from build123d import *

# Parameters (mm, degrees)
EXTRUDE_THIN1_DEPTH = 20
CHAMFER1_SIZE       = 0.3
CUT_EXTRUDE1_REACH  = 53.386
CUT_EXTRUDE2_REACH  = 55.39
SKETCH3_R           = 1.75


with BuildPart() as part:
    # Sketch1 → Extrude-Thin1 (new body)
    with BuildSketch(Plane.XY):
        Polygon((0, 45.5), (0, 0), (24.5, 0), (24.5, 5), (5, 5), (5, 45.5), align=None)
    extrude(amount=EXTRUDE_THIN1_DEPTH)

    # Chamfer1
    chamfer1_edges = [part.edges().sort_by_distance(p)[0] for p in [
        (14.75, 5, 20),
        (5, 25.25, 20),
        (2.5, 45.5, 20),
        (0, 22.75, 20),
        (0, 22.75, 0),
        (2.5, 45.5, 0),
        (5, 25.25, 0),
        (14.75, 5, 0),
        (24.5, 2.5, 0),
        (24.5, 2.5, 20),
        (0, 0, 10),
        (0, 45.5, 10),
        (5, 45.5, 10),
        (5, 5, 10),
        (24.5, 5, 10),
    ]]
    chamfer(chamfer1_edges, length=CHAMFER1_SIZE)

    # Sketch2 → Cut-Extrude1 (cut, up to next)
    with BuildSketch(Plane(origin=(0, 5, 0), x_dir=(1, 0, 0), z_dir=(0, 1, 0)), mode=Mode.PRIVATE) as cut_extrude1_sk1:
        with BuildLine():
            Line((9.5, -8.25), (19.5, -8.25))
            ThreePointArc((19.5, -8.25), (21.25, -10), (19.5, -11.75))
            Line((19.5, -11.75), (9.5, -11.75))
            ThreePointArc((9.5, -11.75), (7.75, -10), (9.5, -8.25))
        make_face()
    cut_extrude1_tool1 = extrude(cut_extrude1_sk1.sketch, amount=-CUT_EXTRUDE1_REACH, mode=Mode.PRIVATE) & part.part
    add(cut_extrude1_tool1.solids().sort_by_distance((14.5, 5, 10))[0], mode=Mode.SUBTRACT)

    # Sketch3 → Cut-Extrude2 (cut, up to next)
    with BuildSketch(Plane(origin=(5, 0, 0), x_dir=(0, 0, -1), z_dir=(1, 0, 0)), mode=Mode.PRIVATE) as cut_extrude2_sk1:
        with Locations(Location((-15, 40.5, 0), (0, 0, 90))):
            Circle(SKETCH3_R)
    cut_extrude2_tool1 = extrude(cut_extrude2_sk1.sketch, amount=-CUT_EXTRUDE2_REACH, mode=Mode.PRIVATE) & part.part
    # Sketch3 → Cut-Extrude2 (cut, up to next)
    with BuildSketch(Plane(origin=(5, 0, 0), x_dir=(0, 0, -1), z_dir=(1, 0, 0)), mode=Mode.PRIVATE) as cut_extrude2_sk2:
        with Locations(Location((-15, 30.5, 0), (0, 0, 90))):
            Circle(SKETCH3_R)
    cut_extrude2_tool2 = extrude(cut_extrude2_sk2.sketch, amount=-CUT_EXTRUDE2_REACH, mode=Mode.PRIVATE) & part.part
    # Sketch3 → Cut-Extrude2 (cut, up to next)
    with BuildSketch(Plane(origin=(5, 0, 0), x_dir=(0, 0, -1), z_dir=(1, 0, 0)), mode=Mode.PRIVATE) as cut_extrude2_sk3:
        with Locations(Location((-5, 30.5, 0), (0, 0, 90))):
            Circle(SKETCH3_R)
    cut_extrude2_tool3 = extrude(cut_extrude2_sk3.sketch, amount=-CUT_EXTRUDE2_REACH, mode=Mode.PRIVATE) & part.part
    # Sketch3 → Cut-Extrude2 (cut, up to next)
    with BuildSketch(Plane(origin=(5, 0, 0), x_dir=(0, 0, -1), z_dir=(1, 0, 0)), mode=Mode.PRIVATE) as cut_extrude2_sk4:
        with Locations(Location((-5, 40.5, 0), (0, 0, 90))):
            Circle(SKETCH3_R)
    cut_extrude2_tool4 = extrude(cut_extrude2_sk4.sketch, amount=-CUT_EXTRUDE2_REACH, mode=Mode.PRIVATE) & part.part
    add(cut_extrude2_tool1.solids().sort_by_distance((5, 40.5, 15))[0], mode=Mode.SUBTRACT)
    add(cut_extrude2_tool2.solids().sort_by_distance((5, 30.5, 15))[0], mode=Mode.SUBTRACT)
    add(cut_extrude2_tool3.solids().sort_by_distance((5, 30.5, 5))[0], mode=Mode.SUBTRACT)
    add(cut_extrude2_tool4.solids().sort_by_distance((5, 40.5, 5))[0], mode=Mode.SUBTRACT)


solid = part.part
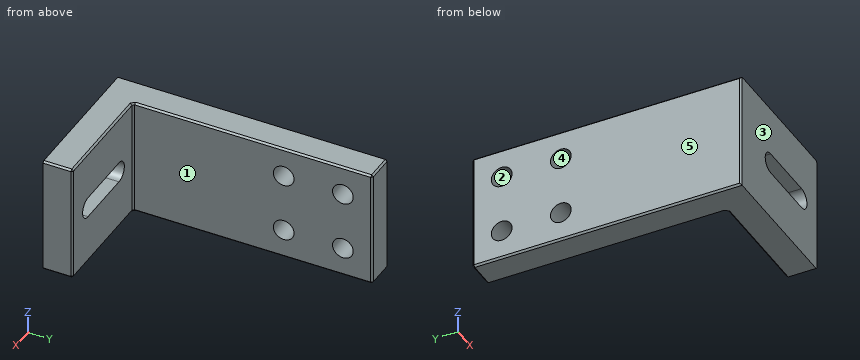
CAD build for the part. Positions are in the model's coordinates, mm. Face numbers are marked on the shaded views. A direction names the side the tool comes from. Give positions to 0.01 mm unless a question says otherwise; leave off trailing zeros. Write each loop counter-clockwise with the first axis right and the second up, starting at its lowest first coordinate (ties: lowest second). Pieces come first, ordered by that corner, then holes. Notation, with made-up numbers: (29, 46) - (52, 46) arc R10 cw to (52, 62) - close; hole circle Ø2 at (-8, 55.25). An arc over 180 degrees is marked (long way). Put each result on its own line as item: value.
(1) Tool access for the marked faces 1 and 2: list every direction of +Z, -Z, +X, -X, +Y, -Y with a clear straight run to the whole face (end or side of a thin tool).
Working result:
face 1: +Z, -Z, +X, +Y
face 2: +X, -X
(2) Saw through at B-B (y = 30.5). List the corners of the cut face in (x, z), then the cut area to 3 significant figures.
Working result:
outline: (0, 0.3) - (0.3, 0) - (4.7, 0) - (5, 0.3) - (5, 3.25) - (0, 3.25) - close; (0, 6.75) - (5, 6.75) - (5, 13.25) - (0, 13.25) - close; (0, 16.75) - (5, 16.75) - (5, 19.7) - (4.7, 20) - (0.3, 20) - (0, 19.7) - close
area: 64.8 mm^2
(3) Pull direction Y, two halves, no side cores. Call the marked faces 3, 4 and 5: released by +Y, released by -Y, zero draft, split by the parting line, or undercut.
Working result:
face 3: released by -Y
face 4: undercut
face 5: zero draft
(4) Wall check: L1, parallel to Z at x = 2.2, y = 30.5; L2, parallel to Y at x = 2.25, z = 3.5; L3, parallel to X at y = 14, z = 1. Give the ranges that are in metal, low to high.
Working result:
L1: 0 to 3.25, 6.75 to 13.25, 16.75 to 20
L2: 0 to 29.6, 31.4 to 39.6, 41.4 to 45.5
L3: 0 to 5
(5) Saw through at D-D (z = 15). List the corners of the cut face in (x, y).
Working result:
outline: (0, 0.3) - (0.3, 0) - (24.5, 0) - (24.5, 4.7) - (24.2, 5) - (5.3, 5) - (5, 5.3) - (5, 28.75) - (0, 28.75) - close; (0, 32.25) - (5, 32.25) - (5, 38.75) - (0, 38.75) - close; (0, 42.25) - (5, 42.25) - (5, 45.2) - (4.7, 45.5) - (0.3, 45.5) - (0, 45.2) - close
(6) Saw through at C-C (x = 3.5). List the corners of the cut face in (y, z).
Working result:
outline: (0, 0) - (45.2, 0) - (45.5, 0.3) - (45.5, 19.7) - (45.2, 20) - (0, 20) - close; hole circle Ø3.5 at (30.5, 5); hole circle Ø3.5 at (30.5, 15); hole circle Ø3.5 at (40.5, 5); hole circle Ø3.5 at (40.5, 15)
(7) Saw through at A-A (z = 10). List the corners of the cut face in (x, y).
Working result:
outline: (0, 0.3) - (0.3, 0) - (7.75, 0) - (7.75, 5) - (5.3, 5) - (5, 5.3) - (5, 45.2) - (4.7, 45.5) - (0.3, 45.5) - (0, 45.2) - close; (21.25, 0) - (24.5, 0) - (24.5, 4.7) - (24.2, 5) - (21.25, 5) - close
(8) Drop flat-ended pins along their axis: pin 1 Ø4.5 at (y, z) = (40.5, 5) entering from +X; pin 2 Ø10 at (x, z) = (20, 11) entering from +Y. Give the stop position or say it passes through.
Working result:
pin 1: x = 5
pin 2: y = 5
